Check sheet for the modelled part. Datum: model origin and axes. Units: mm. A direction names the side the tool comes from. Coordinates: 2 decimals unless noted, no trailing zeros. Order: outer loops, then holes, each group sorted by start corner. A loop starts at its lowest first (then second) coordinate and runs counter-clockwise, first axis right, second up.
from build123d import *

# Parameters (mm, degrees)
T_SLOT_BASE_DEPTH      = 45
CENTRE_BORE_SKETCH_R   = 10
CENTRE_BORE_20_DEPTH   = 45
CLEVIS_LUG_1_PROFILE_R = 6
CLEVIS_LUG_1_DEPTH     = 12
CLEVIS_START           = -12
CLEVIS_LUG_2_PROFILE_R = 6
CLEVIS_LUG_2_DEPTH     = 12


with BuildPart() as part:
    # T-Slot Base Profile → T-Slot Base (new body)
    with BuildSketch(Plane.XY):
        Polygon((-20, 0), (-42.5, 0), (-42.5, 25), (42.5, 25), (42.5, 0), (20, 0), (20, 10), (-20, 10), align=None)
    extrude(amount=T_SLOT_BASE_DEPTH)

    # Centre Bore Sketch → Centre Bore Ø20 (cut)
    with BuildSketch(Plane(origin=(0, 25, 0), x_dir=(1, 0, 0), z_dir=(0, 1, 0))):
        with Locations(Location((0, -22.5, 0), (0, 0, 270))):
            Circle(CENTRE_BORE_SKETCH_R)
    extrude(amount=-CENTRE_BORE_20_DEPTH, mode=Mode.SUBTRACT)

    # Clevis Lug 1 Profile → Clevis Lug 1 (add)
    with BuildSketch(Plane.ZY.offset(42.5)):
        with BuildLine():
            Line((0, 25), (45, 25))
            Line((45, 25), (37.159683171, 61.177056708))
            ThreePointArc((37.159683171, 61.177056708), (22.5, 73), (7.840316829, 61.177056708))
            Line((7.840316829, 61.177056708), (0, 25))
        make_face()
        with Locations((22.5, 58)):
            Circle(CLEVIS_LUG_1_PROFILE_R, mode=Mode.SUBTRACT)
    extrude(amount=-CLEVIS_LUG_1_DEPTH)

    # Clevis Lug 2 Profile → Clevis Lug 2 (add)
    with BuildSketch(Plane(origin=(42.5, 0, 0), x_dir=(0, 0, -1), z_dir=(1, 0, 0)).offset(CLEVIS_START)):
        with BuildLine():
            Line((-37.159683171, 61.177056708), (-45, 25))
            Line((-45, 25), (0, 25))
            Line((0, 25), (-7.840316829, 61.177056708))
            ThreePointArc((-7.840316829, 61.177056708), (-22.5, 73), (-37.159683171, 61.177056708))
        make_face()
        with Locations(Location((-22.5, 58, 0), (0, 0, 180))):
            Circle(CLEVIS_LUG_2_PROFILE_R, mode=Mode.SUBTRACT)
    extrude(amount=CLEVIS_LUG_2_DEPTH)


solid = part.part
(1) Cross-section at C-C (y = 12). Enter the section's corners in (x, z).
Filled in:
outline: (-42.5, 0) - (42.5, 0) - (42.5, 45) - (-42.5, 45) - close; hole circle Ø20 at (0, 22.5)
(2) Cross-section at D-D (y = 58). Enter the section's corners in (x, z).
Filled in:
outline: (-42.5, 7.15) - (-30.5, 7.15) - (-30.5, 16.5) - (-42.5, 16.5) - close; (-42.5, 28.5) - (-30.5, 28.5) - (-30.5, 37.85) - (-42.5, 37.85) - close; (30.5, 7.15) - (42.5, 7.15) - (42.5, 16.5) - (30.5, 16.5) - close; (30.5, 28.5) - (42.5, 28.5) - (42.5, 37.85) - (30.5, 37.85) - close
(3) Cross-section at B-B (z = 22.5). Enter the section's corners in (x, y), and give its area (3 significant figures).
Filled in:
outline: (-42.5, 0) - (-20, 0) - (-20, 10) - (-10, 10) - (-10, 25) - (-30.5, 25) - (-30.5, 52) - (-42.5, 52) - close; (-42.5, 64) - (-30.5, 64) - (-30.5, 73) - (-42.5, 73) - close; (10, 10) - (20, 10) - (20, 0) - (42.5, 0) - (42.5, 52) - (30.5, 52) - (30.5, 25) - (10, 25) - close; (30.5, 64) - (42.5, 64) - (42.5, 73) - (30.5, 73) - close
area: 2,290 mm2
(4) Release check for a two-part mould opening along Y. For faces 4 (the cylindrical face through (36.416, 57.736, 16.506)), 5 (the cylindrical face through (3, 17.6, 32.04)), 6 (the flat face through (36.416, 43.342, 41.025)) record: +Y half, -Y half, draft (parallel to the pull), parting line (faces both ways), or undercut.
Filled in:
face 4: undercut
face 5: draft
face 6: +Y half
(5) Go/stop test with flat-tipped pins: P1, Ø4, axis at x = -15, z = 38.5, coming from the +Y side; P2, Ø11, axis at y = 58, z = 22.5, coming from the -X side; P3, Ø8, axis at x = 30.5, y = 46, coming from the +Z side. Record where each tip stops, or that it passes through.
Filled in:
P1: stops at y = 25
P2: passes through
P3: stops at z = 41.32
(6) Tool access check on faces 1 (the flat face through (0, 10, 12)), 2 (the cylindrical face through (-36.584, 72.997, 22.785)), 3 (the flat face through (-30.5, 44, 22)). Record the directions out of +Z, -Z, +X, -X, +Y, -Y that give a thin tool (end or side, any length) a straight path to the whole face; none if there is none.
Filled in:
face 1: +Z, -Z, -Y
face 2: +X, -X, +Y
face 3: +Z, -Z, +Y
(7) Thickness scan on probe 1 along X at (y, z) = (36, 41); probe 2 along X at (y, z) = (15.75, 22.5); probe 3 along Y at (x, z) = (35, 22). Record the ranges inside material, lowest first.
Filled in:
probe 1: x = -42.5 to -30.5, 30.5 to 42.5
probe 2: x = -42.5 to -10, 10 to 42.5
probe 3: y = 0 to 52.02, 63.98 to 72.99
(8) Cross-section at A-A (x = 0). Enter the section's corners in (y, z).
Filled in:
outline: (10, 0) - (25, 0) - (25, 12.5) - (10, 12.5) - close; (10, 32.5) - (25, 32.5) - (25, 45) - (10, 45) - close
